For this review, take the finished solid that the model builds, in its own axes (mm). Face numbers are marked on the shaded views. A direction names the side the tool comes from. Give positions to 0.01 mm unless a question says otherwise; leave off trailing zeros. Order: outer loops, then holes, each group sorted by start corner. A loop starts at its lowest first (then second) coordinate and runs counter-clockwise, first axis right, second up.
Item 1: Consider section C-C (y = 4.25). Give the boundary of the cut face in (x, z).
Item 2: Consider section A-A (x = 4.5). Give the boundary of the cut face in (y, z), plus the area to 3 significant figures.
Item 3: Consider section B-B (y = 0). Give the boundary of the cut face in (x, z).
Item 4: Consider section D-D (z = 0.25). Give the boundary of the cut face in (x, y), plus the area to 3 significant figures.
Item 5: For P1, Ø4, axis at x = 1.5, y = 0, coming from the -Z side, flat-tipped, find the tip position at first contact; note if it passes through.
Item 6: Machinability: for the marked faces 1, 2 and 3, which of the approach directions +Z, -Z, +X, -X, +Y, -Y give a long, thin tool a straight path to every point of the face, cutting with its end or side? Answer none if there is none.
Item 7: For probe 1 along X at (y, z) = (4.25, 0.35); probe 2 along X at (y, z) = (0, 0.7); probe 3 along X at (y, z) = (-0.75, 0.6), list the stretches that pass through material, from the lowest coordinate up.
Item 8: The part is to be moulded in two halves that separate along X. For the marked faces 4, 5, 6 and 7, say which applies: released by +X, released by -X, zero draft, split by the parting line, or undercut.
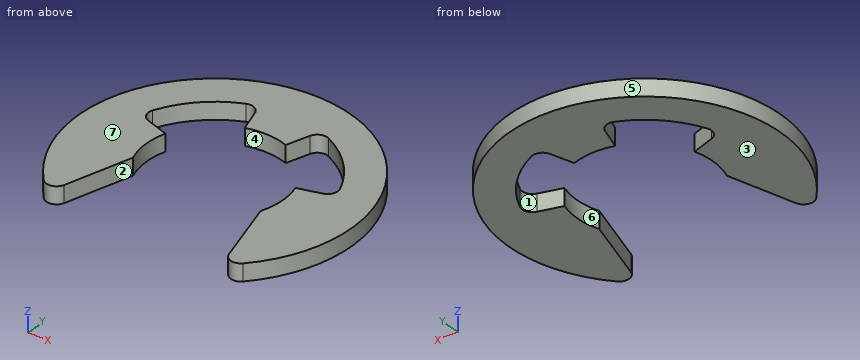
```python
from build123d import *

# Parameters (mm, degrees)
EXTRUDE1_DEPTH = 1


with BuildPart() as part:
    # Sketch1 → Extrude1 (new body)
    with BuildSketch(Plane.XY):
        with BuildLine():
            Line((3.75, -1.391941091), (4.843037844, -5.203817057))
            ThreePointArc((4.843037844, -5.203817057), (5.280177605, -5.621964438), (5.859237689, -5.446956371))
            ThreePointArc((5.859237689, -5.446956371), (0, 8), (-5.859237689, -5.446956371))
            ThreePointArc((-5.859237689, -5.446956371), (-5.280177605, -5.621964438), (-4.843037844, -5.203817057))
            Line((-4.843037844, -5.203817057), (-3.75, -1.391941091))
            ThreePointArc((-3.75, -1.391941091), (-3.998276385, -0.11741359), (-3.825219024, 1.169486819))
            Line((-3.825219024, 1.169486819), (-5.13206986, 1.569031215))
            ThreePointArc((-5.13206986, 1.569031215), (-5.501268007, 1.891044768), (-5.507385374, 2.380904521))
            ThreePointArc((-5.507385374, 2.380904521), (-4.261112254, 4.224088347), (-2.428874258, 5.486398622))
            ThreePointArc((-2.428874258, 5.486398622), (-1.938979773, 5.484556266), (-1.613756661, 5.11818224))
            Line((-1.613756661, 5.11818224), (-1.202823198, 3.814867803))
            ThreePointArc((-1.202823198, 3.814867803), (0, 4), (1.202823198, 3.814867803))
            Line((1.202823198, 3.814867803), (1.613756661, 5.11818224))
            ThreePointArc((1.613756661, 5.11818224), (1.938979773, 5.484556266), (2.428874258, 5.486398622))
            ThreePointArc((2.428874258, 5.486398622), (4.261112254, 4.224088347), (5.507385374, 2.380904521))
            ThreePointArc((5.507385374, 2.380904521), (5.501268007, 1.891044768), (5.13206986, 1.569031215))
            Line((5.13206986, 1.569031215), (3.825219024, 1.169486819))
            ThreePointArc((3.825219024, 1.169486819), (3.998276385, -0.11741359), (3.75, -1.391941091))
        make_face()
    extrude(amount=EXTRUDE1_DEPTH)


solid = part.part
```
Resolved:
1. outline: (-6.78, 0) - (-4.24, 0) - (-4.24, 1) - (-6.78, 1) - close; (-1.34, 0) - (1.34, 0) - (1.34, 1) - (-1.34, 1) - close; (4.24, 0) - (6.78, 0) - (6.78, 1) - (4.24, 1) - close
2. outline: (-4.01, 0) - (1.38, 0) - (1.38, 1) - (-4.01, 1) - close; (3.97, 0) - (6.61, 0) - (6.61, 1) - (3.97, 1) - close
2. area: 8.03 mm2
3. outline: (-8, 0) - (-4, 0) - (-4, 1) - (-8, 1) - close; (4, 0) - (8, 0) - (8, 1) - (4, 1) - close
4. outline: (-5.86, -5.45) arc R0.6 ccw to (-4.84, -5.2) - (-3.75, -1.39) arc R4 cw to (-3.83, 1.17) - (-5.13, 1.57) arc R0.6 cw to (-5.51, 2.38) arc R6 cw to (-2.43, 5.49) arc R0.6 cw to (-1.61, 5.12) - (-1.2, 3.81) arc R4 cw to (1.2, 3.81) - (1.61, 5.12) arc R0.6 cw to (2.43, 5.49) arc R6 cw to (5.51, 2.38) arc R0.6 cw to (5.13, 1.57) - (3.83, 1.17) arc R4 cw to (3.75, -1.39) - (4.84, -5.2) arc R0.6 ccw to (5.86, -5.45) arc R8 ccw (long way) to start
4. area: 90.4 mm2
5. P1: passes through
6. face 1: +Z, -Z
6. face 2: +Z, -Z, -Y
6. face 3: -Z, +X, -X, +Y, -Y
7. probe 1: x = -6.78 to -4.24, -1.34 to 1.34, 4.24 to 6.78
7. probe 2: x = -8 to -4, 4 to 8
7. probe 3: x = -7.96 to -3.93, 3.93 to 7.96
8. face 4: undercut
8. face 5: split by the parting line
8. face 6: undercut
8. face 7: zero draft
